Geometry check sheet. Reference: the model listing, model coordinates, mm. A direction names the side the tool comes from. Give positions to 0.01 mm unless a question says otherwise; leave off trailing zeros. Order: outer loops, then holes, each group sorted by start corner. A loop starts at its lowest first (then second) coordinate and runs counter-clockwise, first axis right, second up. Notation, with made-up numbers: M 62.5,41 L 83.5,41 A27 cw 83.5,71 Z; hole C -6.75,51 d9. An arc over 180 degrees is marked long. Put each result on its own line as item: value. Start each with the question number.
Q1. Section check C-C on x = -15. Record the cut outline in (y, z).
Q2. Mould release check, pull along X, two halves, no side actions. Record for faces 4 (the cylindrical face through (21.146, 8.676, 7.338)), 5 (the flat face through (22, -12.5, 5)), 6 (the flat face through (-5, 10, 5)): +X half, -X half, draft (parallel to the pull), parting line (faces both ways), or undercut.
Q3. Section check B-B on z = 2.5. Record the cut outline in (x, y), then the cut area to 3 significant figures.
Q4. Section check A-A on x = 45. Record the cut outline in (y, z).
Q5. Material ranges on L1, parallel to X at y = -3.75, z = 5; L2, parallel to X at y = -7.75, z = 1.5; L3, parallel to Y at x = 45, z = 7.25, recorded low to high.
Q6. Section check D-D on z = 8.75. Record the cut outline in (x, y), then the cut area to 3 significant figures.
Q7. Access from +Z, -Z, +X, -X, +Y, -Y to the whole of each face (thin tool, end or side, straight path). Record for faces 1 (the flat face through (-27, -7.5, 5)), 2 (the flat face through (-27, 7.5, 5)), 3 (the flat face through (43, 6, 4.6)).
Q8. Go/stop test with flat-tipped pins: pin 1 (2.5 mm diameter, centred on x = 20.5, y = 7.5, fed in from -Z); pin 2 (5 mm diameter, centred on x = -24, z = 5, fed in from +Y); pin 3 (2 mm diameter, centred on x = -33.5, z = 8, fed in from -Y). Record where each tip stops, or that it passes through.
```python
from build123d import *

# Parameters (mm, degrees)
SKETCH1_W                                        = 100
SKETCH1_H                                        = 25
BOSS_EXTRUDE1_DEPTH                              = 10
CUT_EXTRUDE1_DEPTH                               = 53.5
CUT_EXTRUDE1_DEPTH_BACK                          = 53.5
SKETCH2_W                                        = 45
SKETCH2_H                                        = 5
HOLE_FOR_SOCKET_HEAD_CAP_SCREW_TYPE1_D           = 4.5
HOLE_FOR_SOCKET_HEAD_CAP_SCREW_TYPE1_CBORE_D     = 8
HOLE_FOR_SOCKET_HEAD_CAP_SCREW_TYPE1_CBORE_DEPTH = 4.6
M4_TAPPED_HOLE1_D                                = 3.3


with BuildPart() as part:
    # Sketch1 → Boss-Extrude1 (new body)
    with BuildSketch(Plane.XY):
        Rectangle(SKETCH1_W, SKETCH1_H)
    extrude(amount=BOSS_EXTRUDE1_DEPTH)

    # Sketch2 → Cut-Extrude1 (cut, two sides: drawn at the far end of the back side and taken through both)
    with BuildSketch(Plane(origin=(0, 0, 0), x_dir=(-1, 0, 0), z_dir=(0, 0, -1)).offset(-CUT_EXTRUDE1_DEPTH_BACK)):
        with Locations((27.5, 10)):
            Rectangle(SKETCH2_W, SKETCH2_H)
        with Locations((27.5, -10)):
            Rectangle(SKETCH2_W, SKETCH2_H)
    extrude(amount=CUT_EXTRUDE1_DEPTH + CUT_EXTRUDE1_DEPTH_BACK, mode=Mode.SUBTRACT)

    # Hole for socket head cap screw, type1 (through all)
    with Locations(Plane(origin=(0, 0, 0), x_dir=(-1, 0, 0), z_dir=(0, 0, -1))):
        with Locations((-19, -8), (-19, 8), (-45, 8), (-45, -8)):
            CounterBoreHole(HOLE_FOR_SOCKET_HEAD_CAP_SCREW_TYPE1_D / 2, HOLE_FOR_SOCKET_HEAD_CAP_SCREW_TYPE1_CBORE_D / 2, HOLE_FOR_SOCKET_HEAD_CAP_SCREW_TYPE1_CBORE_DEPTH)

    # M4 Tapped Hole1 (through all)
    with Locations(Plane(origin=(0, 7.5, 0), x_dir=(1, 0, 0), z_dir=(0, 1, 0))):
        with Locations((-15, -5), (-40, -5)):
            Hole(M4_TAPPED_HOLE1_D / 2)


solid = part.part
```
Results found:
1. outline: M -7.5,0 L 7.5,0 L 7.5,3.35 L -7.5,3.35 Z; M -7.5,6.65 L 7.5,6.65 L 7.5,10 L -7.5,10 Z
2. face 4: undercut
2. face 5: draft
2. face 6: -X half
3. outline: M -50,-7.5 L -5,-7.5 L -5,-12.5 L 50,-12.5 L 50,12.5 L -5,12.5 L -5,7.5 L -50,7.5 Z; hole C 19,-8 d8; hole C 19,8 d8; hole C 45,-8 d8; hole C 45,8 d8
3. area: 1,850 mm^2
4. outline: M -12.5,0 L -12,0 L -12,4.6 L -10.25,4.6 L -10.25,10 L -12.5,10 Z; M -5.75,4.6 L -4,4.6 L -4,0 L 4,0 L 4,4.6 L 5.75,4.6 L 5.75,10 L -5.75,10 Z; M 10.25,4.6 L 12,4.6 L 12,0 L 12.5,0 L 12.5,10 L 10.25,10 Z
5. L1: x = -50 to -41.65, -38.35 to -16.65, -13.35 to 50
5. L2: x = -5 to 15.01, 22.99 to 41.01, 48.99 to 50
5. L3: y = -12.5 to -10.25, -5.75 to 5.75, 10.25 to 12.5
6. outline: M -50,-7.5 L -5,-7.5 L -5,-12.5 L 50,-12.5 L 50,12.5 L -5,12.5 L -5,7.5 L -50,7.5 Z; hole C 19,-8 d4.5; hole C 19,8 d4.5; hole C 45,-8 d4.5; hole C 45,8 d4.5
6. area: 1,990 mm^2
7. face 1: +Z, -Z, -X, -Y
7. face 2: +Z, -Z, -X, +Y
7. face 3: -Z
8. pin 1: stops at z = 4.6
8. pin 2: stops at y = 7.5
8. pin 3: stops at y = -7.5
